Answer from the drawing. Dimensions are ordinates in mm from the lowest x, y and z of the part. Coordinates: 2 decimals unless noted, no trailing zeros. Loops run counter-clockwise (first coordinate to the right, second up) from the corner with the lowest first, then second, coordinate; pieces in that order, holes last. Notation, with made-up numbers: M 31.5,19 L 56.5,19 A36 ccw 56.5,55 Z; hole C 37.25,41.5 d1. An arc over 180 degrees is marked long. Put each result on its own line as item: value.
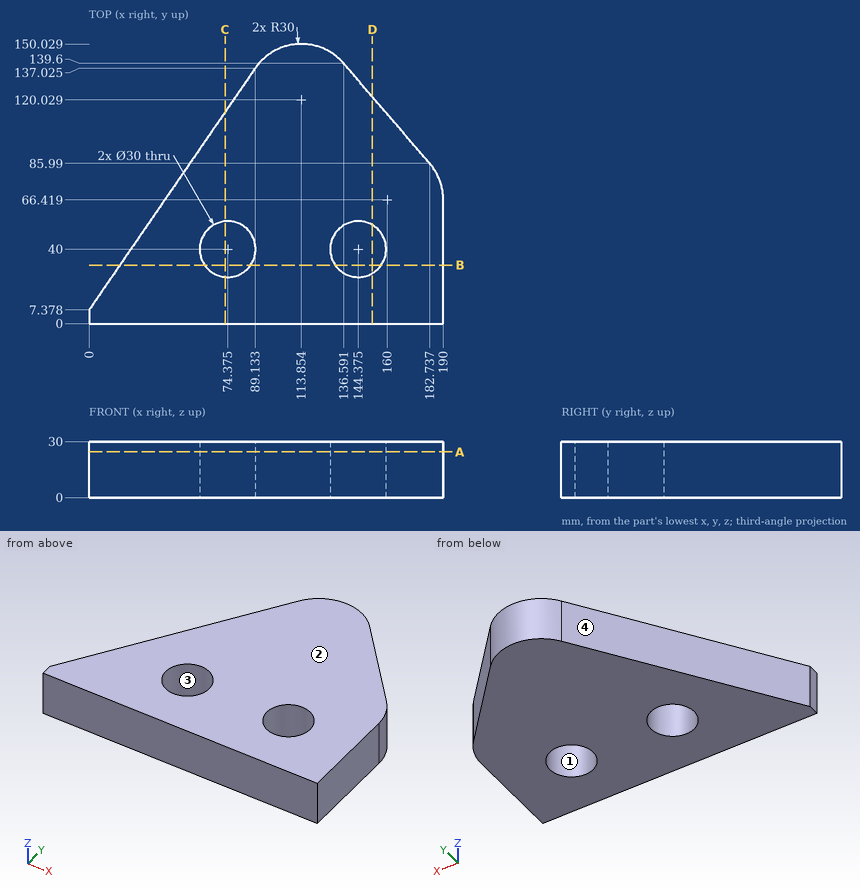
1) Given pin 1 Ø6 at (x, y) = (131.5, 37.5) entering from -Z; pin 2 Ø12 at (y, z) = (86.5, 6) entering from +X; pin 3 Ø1.5 at (y, z) = (134.5, 13) entering from +X (1 decimal), each flat-ended and moving along its own axis, determine where each tip first touches the part or whether it passes through.
Answer list:
pin 1: stops at z = 0
pin 2: stops at x = 186.49
pin 3: stops at x = 141.6
2) Find section C-C, the plane x = 73. Write down the section's boundary in (y, z), plus the area to 3 significant figures.
Answer list:
outline: M 0,0 L 25.06,0 L 25.06,30 L 0,30 Z; M 54.94,0 L 113.56,0 L 113.56,30 L 54.94,30 Z
area: 2,510 mm^2
3) Find section D-D, the plane x = 152. Write down the section's boundary in (y, z).
Answer list:
outline: M 0,0 L 27.08,0 L 27.08,30 L 0,30 Z; M 52.92,0 L 121.7,0 L 121.7,30 L 52.92,30 Z
4) Find section B-B, the plane y = 31.5. Write down the section's boundary in (x, z) (1 decimal), plus the area to 3 significant figures.
Answer list:
outline: M 16.6,0 L 62,0 L 62,30 L 16.6,30 Z; M 86.7,0 L 132,0 L 132,30 L 86.7,30 Z; M 156.7,0 L 190,0 L 190,30 L 156.7,30 Z
area: 3,720 mm^2
5) Straight lines are drawn through the part: line 1 (X direction, y = 40, z = 9) (1 decimal); line 2 (X direction, y = 32, z = 24.5) (1 decimal); line 3 (Y direction, x = 84, z = 19.25) (1 decimal). For each, find the intervals that lie inside material, in ascending order. Write a range as [from, to].
Answer list:
line 1: x = [22.4, 59.4], [89.4, 129.4], [159.4, 190]
line 2: x = [16.9, 61.7], [87.1, 131.7], [157.1, 190]
line 3: y = [0, 28.5], [51.5, 129.6]
6) Find section A-A, the plane z = 24.5. Write down the section's boundary in (x, y) (1 decimal).
Answer list:
outline: M 0,0 L 190,0 L 190,66.4 A30 ccw 182.7,86 L 136.6,139.6 A30 ccw 89.1,137 L 0,7.4 Z; hole C 74.4,40 d30; hole C 144.4,40 d30
7) Determine the mould class of the marked faces 1, 2, 3 and 4 for opening direction Y: released by +Y, released by -Y, zero draft, split by the parting line, or undercut.
Answer list:
face 1: undercut
face 2: zero draft
face 3: undercut
face 4: released by +Y
